Geometry check sheet. Reference: the model listing, model coordinates, mm. A direction names the side the tool comes from. Round coordinates to 2 decimals unless told otherwise and drop trailing zeros. Write each loop counter-clockwise with the first axis right and the second up, starting at its lowest first coordinate (ties: lowest second). Pieces come first, ordered by that corner, then holes. Notation, with made-up numbers: (7.5, 74.5) - (25.5, 74.5) arc R15 cw to (25.5, 89.5) - close; hole circle Ø8 at (29, 3.25). An arc over 180 degrees is marked (long way). Return JSON: item names as keys, results as strings.
```python
from build123d import *

# Parameters (mm, degrees)
NUT_PROFILE_SKETCH_R     = 6.5
FLANGE_DISC_13_DEPTH     = 0.5
SKETCH1_5_R              = 4.5
FLANGE_COLLAR_DEPTH      = 1.5
SKETCH1_6_R              = 2.5
HEX_BODY_DEPTH           = 4.5
TAPER_LOFT_BASE_SKETCH_R = 6.5
TAPER_LOFT_TOP_SKETCH_R  = 4.5
THROUGH_START            = -4.5
BORE_SKETCH_R            = 2.5
THROUGH_BORE_DEPTH       = 4.5


with BuildPart() as part:
    # Nut Profile Sketch → Flange Disc _13 (new body)
    with BuildSketch(Plane(origin=(0, 0, 0), x_dir=(1, 0, 0), z_dir=(0, 1, 0))):
        with Locations(Location((0, 0, 0), (0, 0, 270))):
            Circle(NUT_PROFILE_SKETCH_R)
    extrude(amount=FLANGE_DISC_13_DEPTH)

    # Sketch1_5 → Flange Collar (add)
    with BuildSketch(Plane(origin=(0, 0, 0), x_dir=(1, 0, 0), z_dir=(0, 1, 0))):
        with Locations(Location((0, 0, 0), (0, 0, 270))):
            Circle(SKETCH1_5_R)
    extrude(amount=FLANGE_COLLAR_DEPTH)

    # Sketch1_6 → Hex Body (add)
    with BuildSketch(Plane(origin=(0, 0, 0), x_dir=(1, 0, 0), z_dir=(0, 1, 0))):
        Polygon((-3.14677035, -3.216805304), (1.212449938, -4.333585715), (4.359220287, -1.116780411), (3.14677035, 3.216805304), (-1.212449938, 4.333585715), (-4.359220287, 1.116780411), align=None)
        with Locations(Location((0, 0, 0), (0, 0, 270))):
            Circle(SKETCH1_6_R, mode=Mode.SUBTRACT)
    extrude(amount=HEX_BODY_DEPTH)

    # Taper Loft Base Sketch → Flange Taper Loft section 0
    with BuildSketch(Plane(origin=(0, 0.5, 0), x_dir=(1, 0, 0), z_dir=(0, 1, 0))):
        Circle(TAPER_LOFT_BASE_SKETCH_R)
    # Taper Loft Top Sketch → Flange Taper Loft section 1
    with BuildSketch(Plane(origin=(0, 1.5, 0), x_dir=(1, 0, 0), z_dir=(0, 1, 0))):
        Circle(TAPER_LOFT_TOP_SKETCH_R)
    loft()

    # Bore Sketch → Through Bore (cut)
    with BuildSketch(Plane(origin=(0, 1.5, 0), x_dir=(1, 0, 0), z_dir=(0, 1, 0)).offset(THROUGH_START)):
        with Locations(Location((0, 0, 0), (0, 0, 270))):
            Circle(BORE_SKETCH_R)
    extrude(amount=THROUGH_BORE_DEPTH, mode=Mode.SUBTRACT)


solid = part.part
```
(1) Release check for a two-part mould opening along Z. For faces 1 (the face through (-1, 1.5, 4)), 2 (the face through (-2.44, 2.22, -0.54)), 3 (the face through (3.76, 2.98, -1.02)), 4 (the face through (-3.76, 2.98, 1.02)) record: pulls with the +Z half, pulls with the -Z half, needs draft (parallel to the pull), parting line crosses it, or undercut.
Response values:
{"face 1": "needs draft", "face 2": "undercut", "face 3": "pulls with the -Z half", "face 4": "pulls with the +Z half"}
(2) Access from +Z, -Z, +X, -X, +Y, -Y to the whole of each face (thin tool, end or side, straight path). Record for faces 5 (the face through (-4, 1.5, 1)), 6 (the face through (2.76, 2.98, 2.75)), 7 (the face through (-3, 1.5, -3)).
Response values:
{"face 5": "+Z, -X, +Y", "face 6": "+Z, +X, +Y", "face 7": "-Z, -X, +Y"}
(3) Section check B-B, the plane x = 0. Enter the section's corners in (y, z), plus the area to 3 significant figures.
Response values:
{"outline": "(0, -6.5) - (0.5, -6.5) - (1.5, -4.5) - (1.5, -4.02) - (4.5, -4.02) - (4.5, -2.5) - (0, -2.5) - close; (0, 2.5) - (4.5, 2.5) - (4.5, 4.02) - (1.5, 4.02) - (1.5, 4.5) - (0.5, 6.5) - (0, 6.5) - close", "area": "19.1 mm^2"}
(4) Material ranges on line 1 along X through (y, z) = (2.6, 0); line 2 along Y through (x, z) = (-4, -1.75); line 3 along Z through (x, y) = (0, 3.55), recorded low to high. Write a range as [from, to].
Response values:
{"line 1": "x = [-4.05, -2.5], [2.5, 4.05]", "line 2": "y = [0, 1.5]", "line 3": "z = [-4.02, -2.5], [2.5, 4.02]"}
(5) Gauge pin test, flat ends, axial feed: pin 1 (0.6 mm diameter, centred on x = -0.5, z = 4, fed in from +Y); pin 2 (0.6 mm diameter, centred on x = 1.5, z = -4, fed in from +Y); pin 3 (1.5 mm diameter, centred on x = -0.5, y = 1.5, fed in from -Z); pin 4 (1.5 mm diameter, centred on x = -2.5, y = 1.5, fed in from -Z). Record the tip position at first contact, or that the pin passes through.
Response values:
{"pin 1": "stops at y = 4.5", "pin 2": "stops at y = 1.5", "pin 3": "stops at z = -5.98", "pin 4": "stops at z = -5.49"}
(6) Section check A-A, the plane y = 4. Enter the section's corners in (x, z).
Response values:
{"outline": "(-4.36, -1.12) - (-1.21, -4.33) - (3.15, -3.22) - (4.36, 1.12) - (1.21, 4.33) - (-3.15, 3.22) - close; hole circle Ø5 at (0, 0)"}
